from build123d import *

# Parameters (mm, degrees)
SKETCH_1_W                    = 900
SKETCH_1_H                    = 25
EXTRUDE_1_DEPTH               = 25
SKETCH_2_W                    = 526
SKETCH_2_H                    = 10
EXTRUDE_2_DEPTH               = 35
CUT_EXTRUDE_1_DEPTH           = 902.027191599
CHAMFER_1_SIZE                = 0.5
HOLE_WIZARD_M10_1_D           = 11
HOLE_WIZARD_M10_1_CBORE_D     = 21.48
HOLE_WIZARD_M10_1_CBORE_DEPTH = 6.85
HOLE_WIZARD_M5_1_D            = 5.5
HOLE_WIZARD_M5_1_CBORE_D      = 12.24
HOLE_WIZARD_M5_1_CBORE_DEPTH  = 3.58
HOLE_WIZARD_M5_1_2_AT_2_COUNT = 2
HOLE_WIZARD_M5_1_2_AT_2_PITCH = 34
PATTERN_LINEAR_1_COUNT        = 2
PATTERN_LINEAR_1_PITCH        = 666


with BuildPart() as part:
    # 草图1 → 拉伸1 (new body)
    with BuildSketch(Plane(origin=(0, 0, 0), x_dir=(0, 0, -1), z_dir=(1, 0, 0))):
        with Locations((450, 12.5)):
            Rectangle(SKETCH_1_W, SKETCH_1_H)
    extrude(amount=EXTRUDE_1_DEPTH)

    # 草图2 → 拉伸2 (add)
    with BuildSketch(Plane.ZY):
        with Locations((-450, 5)):
            Rectangle(SKETCH_2_W, SKETCH_2_H)
    extrude(amount=EXTRUDE_2_DEPTH)

    # 草图3 → 切除-拉伸1 (cut, through all)
    with BuildSketch(Plane.XY):
        with BuildLine():
            Line((7.5, 25), (17.5, 25))
            Line((17.5, 25), (17.5, 18.5))
            ThreePointArc((17.5, 18.5), (17.207106781, 17.792893219), (16.5, 17.5))
            Line((16.5, 17.5), (8.5, 17.5))
            ThreePointArc((8.5, 17.5), (7.792893219, 17.792893219), (7.5, 18.5))
            Line((7.5, 18.5), (7.5, 25))
        make_face()
    extrude(amount=-CUT_EXTRUDE_1_DEPTH, mode=Mode.SUBTRACT)

    # 倒角1
    chamfer_1_edges = [part.edges().sort_by_distance(p)[0] for p in [
        (17.5, 25, -450),
        (7.5, 25, -450),
    ]]
    chamfer(chamfer_1_edges, length=CHAMFER_1_SIZE)

    # M10 六角头螺栓的柱形沉头孔1 (through all)
    with Locations(Plane(origin=(-17.5, 10, -675), x_dir=(0, 0, 1), z_dir=(0, 1, 0))):
        with Locations((0, 0), (150.000000001, 0), (300.000000001, 0), (450, 0)):
            CounterBoreHole(HOLE_WIZARD_M10_1_D / 2, HOLE_WIZARD_M10_1_CBORE_D / 2, HOLE_WIZARD_M10_1_CBORE_DEPTH)

    # Hole Wizard M5 _1 (through all)
    with Locations(Plane(origin=(0, 12.5, -887.5), x_dir=(0, 0, -1), z_dir=(-1, 0, 0))):
        with Locations((0, 0), (-875, 0)):
            CounterBoreHole(HOLE_WIZARD_M5_1_D / 2, HOLE_WIZARD_M5_1_CBORE_D / 2, HOLE_WIZARD_M5_1_CBORE_DEPTH)

    # 草图8 → Hole Wizard M5 _1 2 (revolve, cut)
    with BuildSketch(Plane(origin=(0, 14, -800), x_dir=(0, 0, 1), z_dir=(0, 1, 0))):
        Polygon((0, 0), (0, 13.6618073), (2.1, 12.4), (2.1, 10), (2.5, 10), (2.5, 0), align=None)
    hole_wizard_m5_1_2 = revolve(axis=Axis((-6.35, 14, -800), (1, 0, 0)), mode=Mode.SUBTRACT)

    # Hole Wizard M5 _1 2 at 2: Hole Wizard M5 _1 2 ×2
    with Locations(*[(0, 0, i * HOLE_WIZARD_M5_1_2_AT_2_PITCH) for i in range(1, HOLE_WIZARD_M5_1_2_AT_2_COUNT)]):
        add(hole_wizard_m5_1_2, mode=Mode.SUBTRACT)

    # 阵列(线性)1: Hole Wizard M5 _1 2 ×2
    with Locations(*[(0, 0, i * PATTERN_LINEAR_1_PITCH) for i in range(1, PATTERN_LINEAR_1_COUNT)]):
        add(hole_wizard_m5_1_2, mode=Mode.SUBTRACT)

    # 阵列(线性)1 copy 1 sketch → 阵列(线性)1 copy 1 (revolve, cut)
    with BuildSketch(Plane(origin=(0, 14, -100), x_dir=(0, 0, 1), z_dir=(0, 1, 0))):
        Polygon((0, 0), (0, 13.6618073), (2.1, 12.4), (2.1, 10), (2.5, 10), (2.5, 0), align=None)
    revolve(axis=Axis((-6.35, 14, -100), (1, 0, 0)), mode=Mode.SUBTRACT)


solid = part.part
Input: part model. Units: mm. Frame: model coordinates. A direction names the side the tool comes from. Coordinates: 2 decimals unless noted, no trailing zeros. Loops run counter-clockwise (first coordinate to the right, second up) from the corner with the lowest first, then second, coordinate; pieces in that order, holes last.
Q1. Cut plane B-B (z = -636). Output: boundary loops of the cut face in (x, y), then the cut area to 3 significant figures.
Q2. Cut plane A-A (z = -82). Output: boundary loops of the cut face in (x, y).
Q3. Contact query for flat-ended pins moving along their axis: pin 1 (4 mm diameter, centred on y = 13, z = -134, fed in from -X); pin 2 (11 mm diameter, centred on x = -9, y = 4, fed in from -Z); pin 3 (6 mm diameter, centred on x = 13, z = -248.5, fed in from +Y). Output: stop coordinate, or through.
Q4. Material intervals for line 1 (Z direction, x = 13.25, y = 12.5); line 2 (X direction, y = 23.25, z = -673); line 3 (X direction, y = 1.75, z = -675), sorted ascending.
Q5. Draft query along X for faces 4 (the face through (25, 13, -444)), 5 (the face through (1, 0, -444)), 6 (the face through (0, 15, -444)), 7 (the face through (-22, 3.15, -220)). Return one class per face: +X half, -X half, draft (parallel to the pull), parting line (faces both ways), or undercut.
Q6. Set-up query: faces 1 (the face through (-22, 3.15, -370)), 2 (the face through (-17, 10, -454)), 3 (the face through (12, 12, 0)). Return all of +Z, -Z, +X, -X, +Y, -Y with unobstructed straight access to the full face (end or side cutting, diameter ignored); none if empty.
Working result:
1. outline: (-35, 0) - (25, 0) - (25, 25) - (18, 25) - (17.5, 24.5) - (17.5, 18.5) arc R1 cw to (16.5, 17.5) - (8.5, 17.5) arc R1 cw to (7.5, 18.5) - (7.5, 24.5) - (7, 25) - (0, 25) - (0, 10) - (-35, 10) - close
1. area: 900 mm2
2. outline: (0, 0) - (25, 0) - (25, 25) - (18, 25) - (17.5, 24.5) - (17.5, 18.5) arc R1 cw to (16.5, 17.5) - (8.5, 17.5) arc R1 cw to (7.5, 18.5) - (7.5, 24.5) - (7, 25) - (0, 25) - close
3. pin 1: stops at x = 0
3. pin 2: stops at z = -713
3. pin 3: stops at y = 17.5
4. line 1: z = -900 to -890.25, -884.75 to -15.25, -9.75 to 0
4. line 2: x = 0 to 7.5, 17.5 to 25
4. line 3: x = -35 to -23, -12 to 25
5. face 4: +X half
5. face 5: draft
5. face 6: -X half
5. face 7: undercut
6. face 1: +Y
6. face 2: +Z, -Z, -X, +Y
6. face 3: +Z, +X, -X, +Y, -Y
